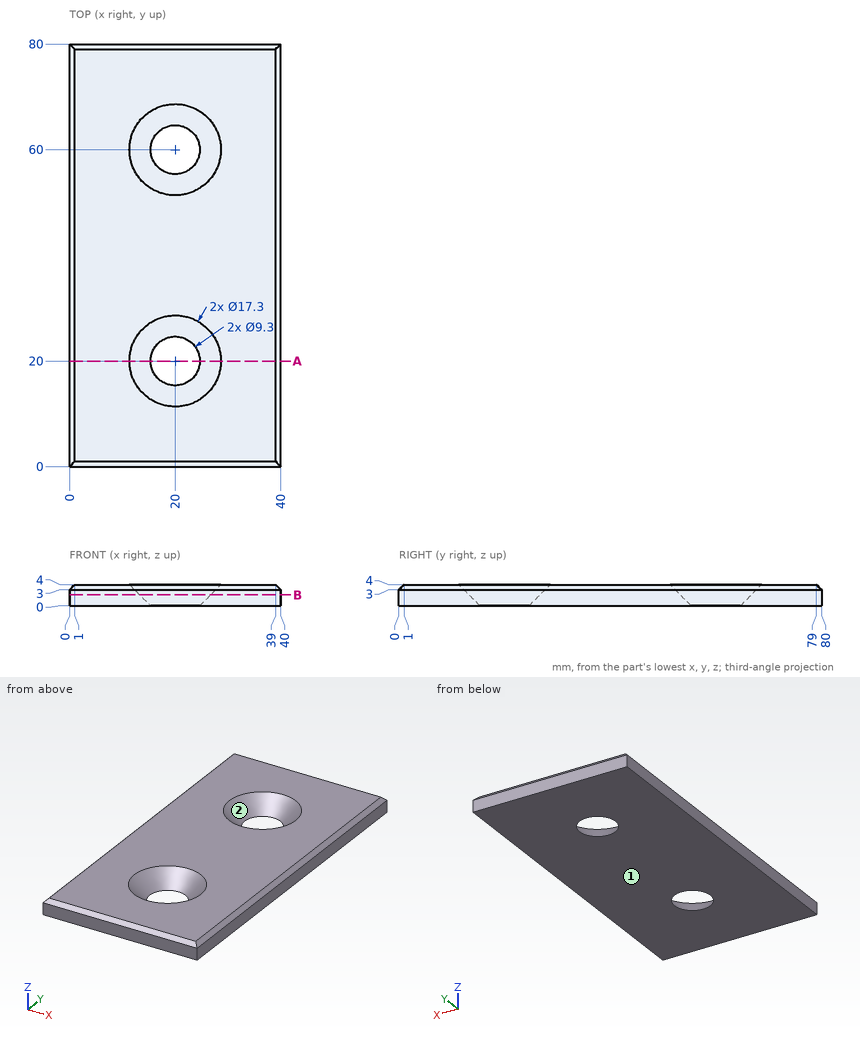
For this review, use the dimensioned drawing (mm, ordinates from the lowest corner) and the shaded views. Coordinates: 2 decimals unless noted, no trailing zeros. Write each loop counter-clockwise with the first axis right and the second up, starting at its lowest first coordinate (ties: lowest second). Pieces come first, ordered by that corner, then holes. Notation, with made-up numbers: (-0.5, 31.25) -> (20.5, 31.25) arc R30 cw to (20.5, 69.25) -> close; hole circle Ø8 at (62.5, 75). An arc over 180 degrees is marked (long way). Write each question's results on one line, items separated by ' | '. Start each with the question number.
(1) For line 1 along Y through (x, z) = (16.5, 2.9); line 2 along Y through (x, z) = (14.5, 2.25); line 3 along Z through (x, y) = (21.5, 67.5), list the stretches that pass through material, from the lowest coordinate up. Write a range as from..to.
(2) The part is to be moulded in two halves that separate along Y. For the marked faces 1 and 2, say which applies: pulls with the +Y half, pulls with the -Y half, needs draft (parallel to the pull), parting line crosses it, or undercut.
(3) Take a section at A-A on y = 20. Write out the cut boundary in (x, z), and give its area (3 significant figures).
(4) Clearance check with a flat-ended pin moving along its axis: P1, Ø6, axis at x = 12, y = 46.5, coming from the -Z side. State where the tip first meets the part, or that it passes through.
(5) Take a section at B-B on z = 2.05. Write out the cut boundary in (x, y).
Results found:
1) line 1: y = 0..13.31, 26.69..53.31, 66.69..80 | line 2: y = 0..15.83, 24.17..55.83, 64.17..80 | line 3: z = 0..3
2) face 1: needs draft | face 2: undercut
3) outline: (0, 0) -> (15.35, 0) -> (11.35, 4) -> (1, 4) -> (0, 3) -> close; (24.65, 0) -> (40, 0) -> (40, 3) -> (39, 4) -> (28.65, 4) -> close | area: 106 mm2
4) P1: stops at z = 0
5) outline: (0, 0) -> (40, 0) -> (40, 80) -> (0, 80) -> close; hole circle Ø13.4 at (20, 20); hole circle Ø13.4 at (20, 60)
